Input: part model. Units: mm. Frame: model coordinates. Coordinates: 2 decimals unless noted, no trailing zeros. Loops run counter-clockwise (first coordinate to the right, second up) from the corner with the lowest first, then second, coordinate; pieces in that order, holes last. Notation, with made-up numbers: M 72,89 L 99,89 A23 cw 99,122 Z; hole C 15.25,-14.5 d7. An arc over 180 degrees is marked long. Use a Markdown table: item, result. Add a question column.
1. Section B-B on x = 67. Output: boundary loops of the cut face in (y, z).
2. Section C-C on y = 44. Output: boundary loops of the cut face in (x, z) (3 decimals), then the cut area to 3 significant figures.
3. Line query: L1, parallel to X at y = 150, z = -2.05; L2, parallel to X at y = 57, z = 0.05; L3, parallel to Y at x = 78, z = -2.35. Output: solid intervals per line, ascending. Write a range as [from, to].
4. Section A-A on z = -0.1. Output: boundary loops of the cut face in (x, y).
```python
from build123d import *

# Parameters (mm, degrees)
BOSS_EXTRUDE1_DEPTH = 3
CHAMFER1_SIZE       = 10


with BuildPart() as part:
    # Sketch1 → Boss-Extrude1 (new, symmetric)
    with BuildSketch(Plane.XY):
        Polygon((0, 170), (0, 0), (130, 0), (130, 10), (60, 170), align=None)
    extrude(amount=BOSS_EXTRUDE1_DEPTH, both=True)

    # Chamfer1
    chamfer1_edges = [part.edges().sort_by_distance(p)[0] for p in [
        (0, 0, 0),
        (0, 170, 0),
    ]]
    chamfer(chamfer1_edges, length=CHAMFER1_SIZE)


solid = part.part
```
Answers below:
| question | item | result |
|---|---|---|
| 1 | outline | M 0,-3 L 154,-3 L 154,3 L 0,3 Z |
| 2 | outline | M 0,-3 L 115.125,-3 L 115.125,3 L 0,3 Z |
| 2 | area | 691 mm² |
| 3 | L1 | x = [0, 68.75] |
| 3 | L2 | x = [0, 109.44] |
| 3 | L3 | y = [0, 128.86] |
| 4 | outline | M 0,10 L 10,0 L 130,0 L 130,10 L 60,170 L 10,170 L 0,160 Z |
